```python
from build123d import *


with BuildPart() as part:
    # Sketch1 → Revolve1 (revolve)
    with BuildSketch(Plane.XY, mode=Mode.PRIVATE) as revolve1_sk:
        Polygon((0, 0), (0, 10), (30, 10), (30, 6), (45, 6), (45, 3), (195, 3), (195, 0), align=None)
    revolve(revolve1_sk.sketch.rotate(Axis((0, 0, 0), (1, 0, 0)), 90), axis=Axis((0, 0, 0), (1, 0, 0)))


solid = part.part
```
Read the model definition and answer for the solid it produces. Units are mm, in the model's axes. A direction names the side the tool comes from. Coordinates: 2 decimals unless noted, no trailing zeros. Write each loop counter-clockwise with the first axis right and the second up, starting at its lowest first coordinate (ties: lowest second). Pieces come first, ordered by that corner, then holes. Notation, with made-up numbers: (83.25, 52) -> (96.25, 52) arc R30 cw to (96.25, 88) -> close; hole circle Ø8 at (-27, 67). An arc over 180 degrees is marked (long way). Return JSON: item names as keys, results as strings.
1. A cutting plane is placed at D-D (x = 96). Determine the outline of the cut face in (y, z), and give its area (3 significant figures).
Found:
{"outline": "circle Ø6 at (0, 0)", "area": "28.3 mm2"}
2. A cutting plane is placed at A-A (y = 0). Determine the outline of the cut face in (x, z), and give its area (3 significant figures).
Found:
{"outline": "(0, -10) -> (30, -10) -> (30, -6) -> (45, -6) -> (45, -3) -> (195, -3) -> (195, 3) -> (45, 3) -> (45, 6) -> (30, 6) -> (30, 10) -> (0, 10) -> close", "area": "1,680 mm2"}
3. Find the intervals of material crossed by line 1 along X through (y, z) = (3.75, 5); line 2 along X through (y, z) = (-0.75, 3); line 3 along Y through (x, z) = (97, -1.5), in increasing order. Write a range as from..to.
Found:
{"line 1": "0..30", "line 2": "0..45", "line 3": "-2.6..2.6"}
4. Each of these flat-tipped pins is pushed along its axis until it touches: P1, Ø6, axis at x = 167.5, y = 0.5, coming from the -Z side; P2, Ø10, axis at x = 118, z = -6.5, coming from the +Y side; P3, Ø5, axis at x = 77, z = -3, coming from the +Y side. Where does it stop, or does it pass through?
Found:
{"P1": "z = -3", "P2": "y = 2.6", "P3": "y = 2.96"}
5. A cutting plane is placed at C-C (x = 39.5). Determine the outline of the cut face in (y, z), and give its area (3 significant figures).
Found:
{"outline": "circle Ø12 at (0, 0)", "area": "113 mm2"}
6. A tool of negligible diameter and unlimited length cuts with its end or side. For faces 1 (the face through (195, 0, 0)), 2 (the face through (37.605, -1.802, 5.723)), from which of +Z, -Z, +X, -X, +Y, -Y can it reach the whole face along a straight path? Write none if from no direction.
Found:
{"face 1": "+Z, -Z, +X, +Y, -Y", "face 2": "+X"}
